For this review, use the dimensioned drawing (mm, ordinates from the lowest corner) and the shaded views. A direction names the side the tool comes from. Coordinates: 2 decimals unless noted, no trailing zeros. Loops run counter-clockwise (first coordinate to the right, second up) from the corner with the lowest first, then second, coordinate; pieces in that order, holes last. Notation, with made-up numbers: (67.25, 73) - (108.25, 73) arc R28 cw to (108.25, 98) - close; hole circle Ø1 at (38, 59.25). An arc over 180 degrees is marked (long way). Answer in a Markdown table with one row per item. Add a question column.
(1) For P1, Ø8, axis at y = 45.5, z = 66.5, coming from the -X side; P2, Ø3, axis at y = 58.5, z = 69, coming from the -X side; P3, Ø5, axis at x = 46.5, z = 19.5, coming from the +Y side; P4, Ø24, axis at y = 50, z = 49, coming from the -X side, all flat-tipped, find the tip position at first contact; note any pin that passes through.
(2) We need section D-D on x = 83. Write out the cut boundary in (y, z), plus the area to 3 significant figures.
(3) We need section A-A on y = 40. Write out the cut boundary in (x, z).
(4) For line 1 along Y through (x, z) = (139, 41); line 2 along Z through (x, y) = (141.5, 56.5), list the stretches that pass through material, from the lowest coordinate up.
(5) Machinability: for the marked faces 1 and 2, which of the approach directions +Z, -Z, +X, -X, +Y, -Y give a long, thin tool a straight path to every point of the face, cutting with its end or side? Answer none if there is none.
(6) We need section C-C on x = 159. Write out the cut boundary in (y, z), plus the area to 3 significant figures.
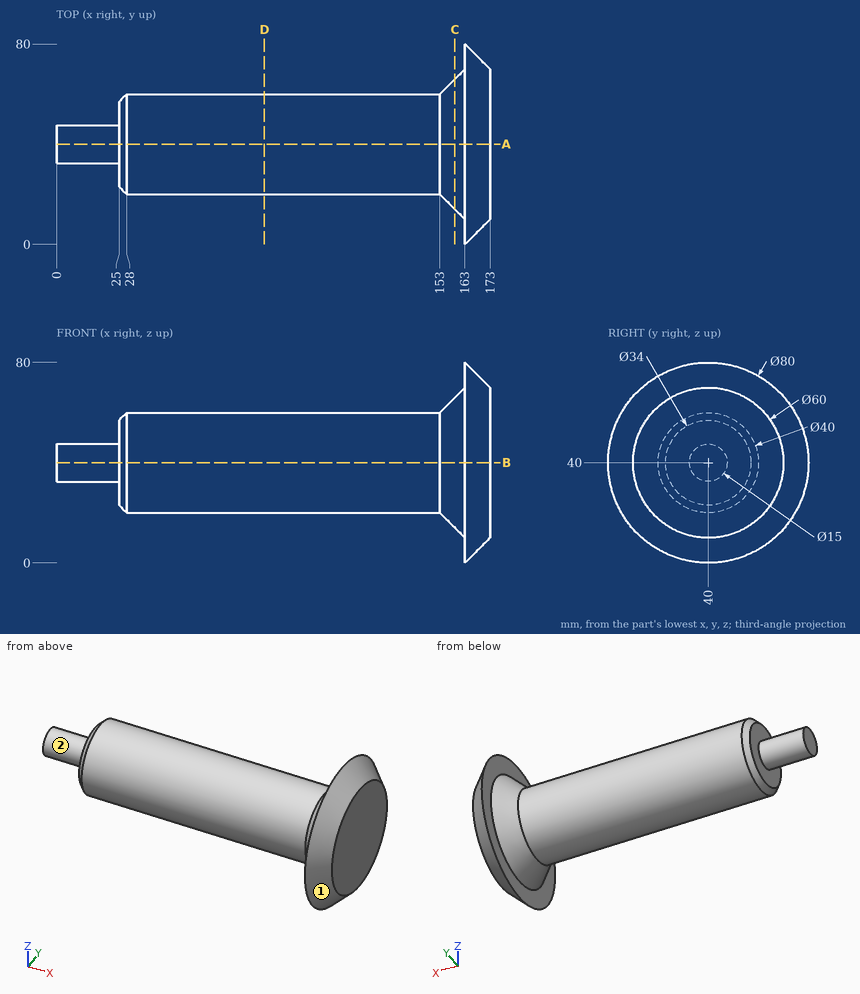
Outcome:
| question | item | result |
|---|---|---|
| 1 | P1 | x = 156.06 |
| 1 | P2 | x = 163 |
| 1 | P3 | y = 48.72 |
| 1 | P4 | x = 0 |
| 2 | outline | circle Ø40 at (40, 40) |
| 2 | area | 1,260 mm² |
| 3 | outline | (0, 32.5) - (25, 32.5) - (25, 23) - (28, 20) - (153, 20) - (163, 10) - (163, 0) - (173, 10) - (173, 70) - (163, 80) - (163, 70) - (153, 60) - (28, 60) - (25, 57) - (25, 47.5) - (0, 47.5) - close |
| 4 | line 1 | 20.03 to 59.97 |
| 4 | line 2 | 28.7 to 51.3 |
| 5 | face 1 | +X |
| 5 | face 2 | -X |
| 6 | outline | circle Ø52 at (40, 40) |
| 6 | area | 2,120 mm² |
